Input: part model. Units: mm. Frame: model coordinates. Round coordinates to 2 decimals unless told otherwise and drop trailing zeros. Order: outer loops, then holes, each group sorted by start corner. A loop starts at its lowest first (then second) coordinate and runs counter-clockwise, first axis right, second up. Notation, with made-up numbers: (-13.5, 61.5) -> (7.5, 61.5) arc R20 ccw to (7.5, 83.5) -> close; hole circle Ø11 at (87.25, -32.5). An arc over 180 degrees is marked (long way). Answer as CSV lines item,"result". Start each with the question number.
1) Section query B-B, the plane x = 13.25. Output: boundary loops of the cut face in (y, z), and give its area (3 significant figures).
2) Section query C-C, the plane y = -8. Output: boundary loops of the cut face in (x, z), and give its area (3 significant figures).
3) First-contact query: P1, Ø5, axis at x = 14, y = -15, coming from the +Z side; P2, Ø2, axis at x = 5, z = -80.5, coming from the +Y side; P3, Ø5, axis at x = 15, y = -10.5, coming from the +Z side; P4, Ø8, axis at x = 14, z = -74, coming from the +Y side. Flat tips, straight axial feed; report the tip coordinate or a pass-through.
4) Section query A-A, the plane z = 108. Output: boundary loops of the cut face in (x, y).
5) Line query: L1, parallel to Z at x = 10.75, y = -15; L2, parallel to Y at x = 4.75, z = -151; L3, parallel to Y at x = 10, z = -44. Output: solid intervals per line, ascending.
```python
from build123d import *

# Parameters (mm, degrees)
EXTRUDE_1_DEPTH = 18.8


with BuildPart() as part:
    # 草图1 → 拉伸-薄壁1 (new body)
    with BuildSketch(Plane(origin=(0, 0, 0), x_dir=(0, 0, -1), z_dir=(1, 0, 0))):
        with BuildLine():
            Line((138.314113207, -107.167648268), (-89.533532193, -83.052342215))
            ThreePointArc((-89.533532193, -83.052342215), (-149.973777418, -15.877541233), (-89.533532193, 51.29725975))
            Line((-89.533532193, 51.29725975), (138.314113207, 75.412565802))
            ThreePointArc((138.314113207, 75.412565802), (239.776222582, -15.877541233), (138.314113207, -107.167648268))
        make_face()
        with BuildLine():
            Line((139.998140985, -91.256518501), (-87.849504415, -67.141212449))
            ThreePointArc((-87.849504415, -67.141212449), (-133.973777418, -15.877541233), (-87.849504415, 35.386129983))
            Line((-87.849504415, 35.386129983), (139.998140985, 59.501436035))
            ThreePointArc((139.998140985, 59.501436035), (223.776222582, -15.877541233), (139.998140985, -91.256518501))
        make_face(mode=Mode.SUBTRACT)
    extrude(amount=EXTRUDE_1_DEPTH)


solid = part.part
```
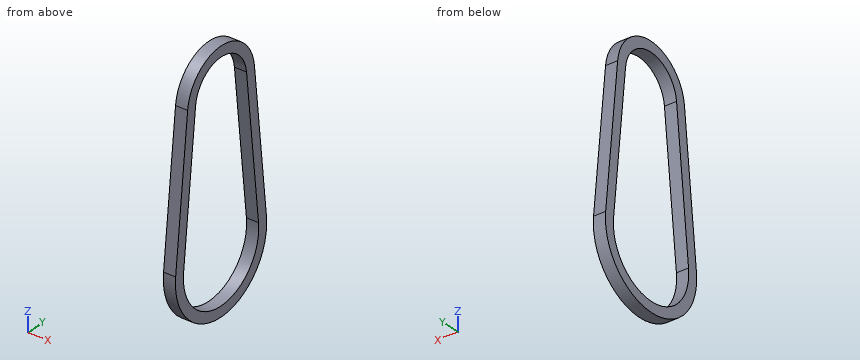
Findings:
1,outline,"(-107.17, -138.31) arc R91.8 ccw (long way) to (75.41, -138.31) -> (51.3, 89.53) arc R67.55 ccw to (-83.05, 89.53) -> close; hole (-91.26, -140) arc R75.8 ccw (long way) to (59.5, -140) -> (35.39, 87.85) arc R51.55 ccw to (-67.14, 87.85) -> close"
1,area,"14,600 mm^2"
2,outline,"(0, -239.44) -> (18.8, -239.44) -> (18.8, -223.37) -> (0, -223.37) -> close; (0, 133.37) -> (18.8, 133.37) -> (18.8, 149.51) -> (0, 149.51) -> close"
2,area,"606 mm^2"
3,P1,"stops at z = 149.97"
3,P2,"stops at y = 69.4"
3,P3,"stops at z = 149.91"
3,P4,"stops at y = 69.03"
4,outline,"(0, -78.4) -> (18.8, -78.4) -> (18.8, -60.64) -> (0, -60.64) -> close; (0, 28.88) -> (18.8, 28.88) -> (18.8, 46.64) -> (0, 46.64) -> close"
5,L1,"z = -239.77 to -223.77, 133.97 to 149.97"
5,L2,"y = -107.63 to -91.62, 59.86 to 75.87"
5,L3,"y = -97.19 to -81.1, 49.34 to 65.43"
